For this review, take the finished solid that the model builds, in its own axes (mm). Round coordinates to 2 decimals unless told otherwise and drop trailing zeros. Write each loop counter-clockwise with the first axis right and the second up, starting at its lowest first coordinate (ties: lowest second). Pieces come first, ordered by that corner, then holes. Notation, with made-up numbers: M -36,64.5 L -6,64.5 A20 ccw -6,77.5 Z; hole C -26,5 d7. An arc over 180 degrees is marked long. Use one line per item in the form item = value. Start each with the question number.
Item 1: Add section B-B (y = 176). State the section outline as (x, z) points.
Item 2: For line 1 (X direction, y = 240, z = 1.05); line 2 (Y direction, x = -170, z = 0.65); line 3 (Y direction, x = -340, z = 0.9), list the stretches that pass through material, from the lowest coordinate up. Write a range as [from, to].
Item 3: For P1, Ø2.5, axis at x = -320, y = -240, coming from the -Z side (3 decimals), flat-tipped, find the tip position at first contact; note if it passes through.
Item 4: Add section A-A (x = 250). State the section outline as (y, z) points.
Item 5: Draft analysis for pull direction X (two halves, no side actions). For faces 1 (the flat face through (-5, 4, 0)), 2 (the cylindrical face through (282.33, 136.59, 1.01)), state which applies: released by +X, released by -X, zero draft, split by the parting line, or undercut.
from build123d import *

# Parameters (mm, degrees)
SKETCH_1_W              = 700
SKETCH_1_H              = 500
EXTRUDE_1_DEPTH         = 2
HOLE_WIZARD_4_5_4_5_1_D = 4.5
SKETCH_4_R              = 35
CUT_EXTRUDE_1_DEPTH     = 10


with BuildPart() as part:
    # 草图1 → 凸台-拉伸1 (new body)
    with BuildSketch(Plane.XY):
        Rectangle(SKETCH_1_W, SKETCH_1_H)
    extrude(amount=EXTRUDE_1_DEPTH)

    # Ø4.5 (4.5) 直径孔1 (through all)
    with Locations(Plane.XY.offset(2)):
        with Locations((320, -240), (-340, 0), (0, -240), (340, 0), (0, 240), (-170, 240), (170, 240), (-170, -240), (170, -240), (-320, 240), (320, 240), (-340, 200), (-340, -200), (340, -200), (340, 200), (-320, -240)):
            Hole(HOLE_WIZARD_4_5_4_5_1_D / 2)

    # 草图4 → 切除-拉伸1 (cut)
    with BuildSketch(Plane.XY.offset(2)):
        with Locations((250, 150)):
            Circle(SKETCH_4_R)
    extrude(amount=-CUT_EXTRUDE_1_DEPTH, mode=Mode.SUBTRACT)


solid = part.part
Calculated:
q1.outline = M -350,0 L 226.57,0 L 226.57,2 L -350,2 Z; M 273.43,0 L 350,0 L 350,2 L 273.43,2 Z
q2.line_1 = [-350, -322.25], [-317.75, -172.25], [-167.75, -2.25], [2.25, 167.75], [172.25, 317.75], [322.25, 350]
q2.line_2 = [-250, -242.25], [-237.75, 237.75], [242.25, 250]
q2.line_3 = [-250, -202.25], [-197.75, -2.25], [2.25, 197.75], [202.25, 250]
q3.P1 = through
q4.outline = M -250,0 L 115,0 L 115,2 L -250,2 Z; M 185,0 L 250,0 L 250,2 L 185,2 Z
q5.face_1 = zero draft
q5.face_2 = undercut
